from build123d import *

# Parameters (mm, degrees)
SKETCH1_R      = 2.25
EXTRUDE1_DEPTH = 6.5
EXTRUDE2_DEPTH = 111.5
SKETCH3_R      = 25
EXTRUDE3_DEPTH = 3
SKETCH4_R      = 7
EXTRUDE4_DEPTH = 27


with BuildPart() as part:
    # Sketch1 → Extrude1 (new body)
    with BuildSketch(Plane.XY):
        with BuildLine():
            Line((-25, -30), (25, -30))
            ThreePointArc((25, -30), (28.535533906, -28.535533906), (30, -25))
            Line((30, -25), (30, 25))
            ThreePointArc((30, 25), (28.535533906, 28.535533906), (25, 30))
            Line((25, 30), (-25, 30))
            ThreePointArc((-25, 30), (-28.535533906, 28.535533906), (-30, 25))
            Line((-30, 25), (-30, -25))
            ThreePointArc((-30, -25), (-28.535533906, -28.535533906), (-25, -30))
        make_face()
        with Locations(Location((-24.748737342, 24.748737342, 0), (0, 0, 180))):
            Circle(SKETCH1_R, mode=Mode.SUBTRACT)
        with Locations(Location((-24.748737342, -24.748737342, 0), (0, 0, 180))):
            Circle(SKETCH1_R, mode=Mode.SUBTRACT)
        with Locations(Location((24.748737342, -24.748737342, 0), (0, 0, 180))):
            Circle(SKETCH1_R, mode=Mode.SUBTRACT)
        with Locations(Location((24.748737342, 24.748737342, 0), (0, 0, 180))):
            Circle(SKETCH1_R, mode=Mode.SUBTRACT)
    extrude(amount=EXTRUDE1_DEPTH)

    # Sketch2 → Extrude2 (add)
    with BuildSketch(Plane.XY.offset(6.5)):
        with BuildLine():
            Line((-19.497474683, -30), (19.497474683, -30))
            Line((19.497474683, -30), (19.497474683, -24.748737342))
            ThreePointArc((19.497474683, -24.748737342), (21.035533906, -21.035533906), (24.748737342, -19.497474683))
            Line((24.748737342, -19.497474683), (30, -19.497474683))
            Line((30, -19.497474683), (30, 19.497474683))
            Line((30, 19.497474683), (24.748737342, 19.497474683))
            ThreePointArc((24.748737342, 19.497474683), (21.035533906, 21.035533906), (19.497474683, 24.748737342))
            Line((19.497474683, 24.748737342), (19.497474683, 30))
            Line((19.497474683, 30), (-19.497474683, 30))
            Line((-19.497474683, 30), (-19.497474683, 24.748737342))
            ThreePointArc((-19.497474683, 24.748737342), (-21.035533906, 21.035533906), (-24.748737342, 19.497474683))
            Line((-24.748737342, 19.497474683), (-30, 19.497474683))
            Line((-30, 19.497474683), (-30, -19.497474683))
            Line((-30, -19.497474683), (-24.748737342, -19.497474683))
            ThreePointArc((-24.748737342, -19.497474683), (-21.035533906, -21.035533906), (-19.497474683, -24.748737342))
            Line((-19.497474683, -24.748737342), (-19.497474683, -30))
        make_face()
    extrude(amount=EXTRUDE2_DEPTH)

    # Sketch3 → Extrude3 (add)
    with BuildSketch(Plane(origin=(0, 0, 0), x_dir=(-1, 0, 0), z_dir=(0, 0, -1))):
        Circle(SKETCH3_R)
    extrude(amount=EXTRUDE3_DEPTH)

    # Sketch4 → Extrude4 (add)
    with BuildSketch(Plane(origin=(0, 0, -3), x_dir=(-1, 0, 0), z_dir=(0, 0, -1))):
        Circle(SKETCH4_R)
    extrude(amount=EXTRUDE4_DEPTH)


solid = part.part
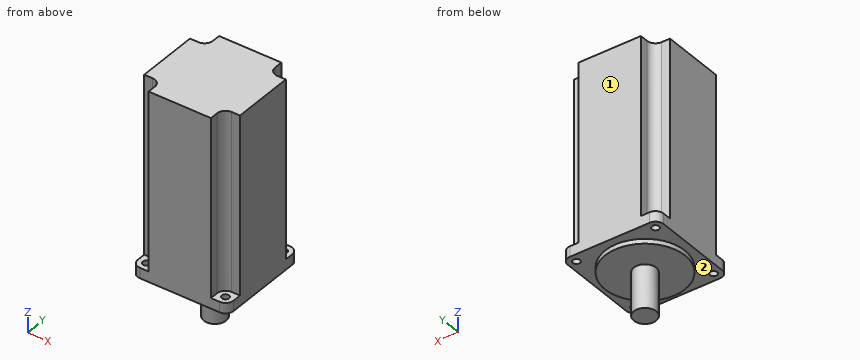
Could you check a few things on this model? Use its own coordinates, in mm. Face numbers are marked on the shaded views. A direction names the side the tool comes from. Coordinates: 2 decimals unless noted, no trailing zeros. Loops run counter-clockwise (first coordinate to the right, second up) from the corner with the lowest first, then second, coordinate; pieces in that order, holes last. Notation, with made-up numbers: (16.5, -0.75) -> (48.5, -0.75) arc R22 cw to (48.5, 32.25) -> close; hole circle Ø11 at (24.25, 39.5). An arc over 180 degrees is marked (long way). Answer in a Markdown table with one row per item.
(1) If I drill on probe 1 along Z at (x, y) = (12.5, -24.5); probe 2 along Y at (x, z) = (-26, 78); probe 3 along Z at (x, y) = (-13, -2), over which ranges is the centre line in solid material (lowest first)?
Results found:
| item | result |
|---|---|
| probe 1 | z = 0 to 118 |
| probe 2 | y = -19.5 to 19.5 |
| probe 3 | z = -3 to 118 |
(2) Imagine slicing it at C-C (z = 108.5). List the corners of the cut face in (x, y) for me.
Results found:
| item | result |
|---|---|
| outline | (-30, -19.5) -> (-24.75, -19.5) arc R5.25 cw to (-19.5, -24.75) -> (-19.5, -30) -> (19.5, -30) -> (19.5, -24.75) arc R5.25 cw to (24.75, -19.5) -> (30, -19.5) -> (30, 19.5) -> (24.75, 19.5) arc R5.25 cw to (19.5, 24.75) -> (19.5, 30) -> (-19.5, 30) -> (-19.5, 24.75) arc R5.25 cw to (-24.75, 19.5) -> (-30, 19.5) -> close |
(3) For the marked faces 1 and 2, which set-ups out of +Z, -Z, +X, -X, +Y, -Y let a thin tool reach every point of the face, with its end or its side?
Results found:
| item | result |
|---|---|
| face 1 | +Z, -Z, +X, -X, +Y |
| face 2 | -Z |
(4) Will these pins go through, and if not, where does the flat tip stop? pin 1 Ø2.5 at (y, z) = (27.5, 57.5) entering from -X; pin 2 Ø1.5 at (y, z) = (23.5, 69.5) entering from +X; pin 3 Ø6 at (x, y) = (-24.75, 24.75) entering from +Z.
Results found:
| item | result |
|---|---|
| pin 1 | stops at x = -19.5 |
| pin 2 | stops at x = 19.89 |
| pin 3 | stops at z = 6.5 |
(5) Imagine slicing it at D-D (x = 13). List the corners of the cut face in (y, z) for me.
Results found:
| item | result |
|---|---|
| outline | (-30, 0) -> (-21.35, 0) -> (-21.35, -3) -> (21.35, -3) -> (21.35, 0) -> (30, 0) -> (30, 118) -> (-30, 118) -> close |
(6) Imagine slicing it at A-A (x = 0). List the corners of the cut face in (y, z) for me.
Results found:
| item | result |
|---|---|
| outline | (-30, 0) -> (-25, 0) -> (-25, -3) -> (-7, -3) -> (-7, -30) -> (7, -30) -> (7, -3) -> (25, -3) -> (25, 0) -> (30, 0) -> (30, 118) -> (-30, 118) -> close |
